```python
from build123d import *

# Parameters (mm, degrees)
SKETCH_1_W                = 82
SKETCH_1_H                = 82
EXTRUDE_1_DEPTH           = 10
SKETCH_4_R                = 10.5
CUT_EXTRUDE_3_DEPTH       = 59.838762733
FILLET_9_R                = 10
HOLE_WIZARD_2_D           = 4.3
HOLE_WIZARD_2_CBORE_D     = 8
HOLE_WIZARD_2_CBORE_DEPTH = 4.6
HOLE_WIZARD_M4_2_D        = 3.3
HOLE_WIZARD_M4_2_DEPTH    = 18.5
HOLE_WIZARD_M4_2_TIP      = 0.991420021
MM_2_D                    = 21.1
HOLE_WIZARD_M4_3_D        = 3.3
HOLE_WIZARD_M6_1_D        = 5
HOLE_WIZARD_M6_2_D        = 5
HOLE_WIZARD_5_0_5_1_D     = 5
HOLE_WIZARD_5_0_5_1_DEPTH = 10
HOLE_WIZARD_5_0_5_1_TIP   = 1.502151548


with BuildPart() as part:
    # 草图1 → 凸台-拉伸1 (new body)
    with BuildSketch(Plane(origin=(0, 0, 0), x_dir=(1, 0, 0), z_dir=(0, 1, 0))):
        Rectangle(SKETCH_1_W, SKETCH_1_H)
    extrude(amount=EXTRUDE_1_DEPTH)

    # 草图4 → 切除-拉伸3 (cut, through all)
    with BuildSketch(Plane(origin=(0, 10, 0), x_dir=(1, 0, 0), z_dir=(0, 1, 0))):
        with Locations(Location((0, -27.5, 0), (0, 0, 270))):
            Circle(SKETCH_4_R)
    extrude(amount=-CUT_EXTRUDE_3_DEPTH, mode=Mode.SUBTRACT)

    # 圆角9
    fillet_9_edges = [part.edges().sort_by_distance(p)[0] for p in [
        (41, 5, 41),
        (-41, 5, 41),
    ]]
    fillet(fillet_9_edges, radius=FILLET_9_R)

    # 打孔尺寸(%根据)开槽圆柱头螺钉的类型2 (through all)
    with Locations(Plane(origin=(0, 10, 0), x_dir=(1, 0, 0), z_dir=(0, 1, 0))):
        with Locations((-16.5, -27.5), (16.5, -27.5)):
            CounterBoreHole(HOLE_WIZARD_2_D / 2, HOLE_WIZARD_2_CBORE_D / 2, HOLE_WIZARD_2_CBORE_DEPTH)

    # M4 螺纹孔2
    with Locations(Plane(origin=(0, 0, -41), x_dir=(-1, 0, 0), z_dir=(0, 0, -1))):
        with Locations((-22.5, 5), (22.5, 5)):
            Hole(HOLE_WIZARD_M4_2_D / 2, depth=HOLE_WIZARD_M4_2_DEPTH)
            with Locations((0, 0, -(HOLE_WIZARD_M4_2_DEPTH + HOLE_WIZARD_M4_2_TIP / 2))):  # 118° drill point
                Cone(0, HOLE_WIZARD_M4_2_D / 2, HOLE_WIZARD_M4_2_TIP, mode=Mode.SUBTRACT)

    # 大小mm 暗销孔2 (through all)
    with Locations(Plane(origin=(0, 10, 0), x_dir=(1, 0, 0), z_dir=(0, 1, 0))):
        with Locations((-25, 13), (25, 13)):
            Hole(MM_2_D / 2)

    # M4 螺纹孔3 (through all)
    with Locations(Plane(origin=(0, 0, 0), x_dir=(-1, 0, 0), z_dir=(0, -1, 0))):
        with Locations((-13.686291501, 24.313708499), (-13.686291501, 1.686291501), (-36.313708499, 1.686291501), (-36.313708499, 24.313708499)):
            hole_wizard_m4_3 = Hole(HOLE_WIZARD_M4_3_D / 2)

    # 镜向2: M4 螺纹孔3 across plane
    add(hole_wizard_m4_3.mirror(Plane(origin=(0, 0, 0), x_dir=(0, 0, 1), z_dir=(1, 0, 0))), mode=Mode.SUBTRACT)

    # M6 螺纹孔1 (through all)
    with Locations(Plane(origin=(0, 10, 0), x_dir=(1, 0, 0), z_dir=(0, 1, 0))):
        with Locations((0, 22)):
            Hole(HOLE_WIZARD_M6_1_D / 2)

    # M6 螺纹孔2 (through all)
    with Locations(Plane(origin=(0, 10, 0), x_dir=(1, 0, 0), z_dir=(0, 1, 0))):
        with Locations((0, -4)):
            Hole(HOLE_WIZARD_M6_2_D / 2)

    # Ø5.0 (5) 直径孔1
    with Locations(Plane(origin=(0, 0, -41), x_dir=(-1, 0, 0), z_dir=(0, 0, -1))):
        with Locations((-32.5, 5), (32.5, 5)):
            Hole(HOLE_WIZARD_5_0_5_1_D / 2, depth=HOLE_WIZARD_5_0_5_1_DEPTH)
            with Locations((0, 0, -(HOLE_WIZARD_5_0_5_1_DEPTH + HOLE_WIZARD_5_0_5_1_TIP / 2))):  # 118° drill point
                Cone(0, HOLE_WIZARD_5_0_5_1_D / 2, HOLE_WIZARD_5_0_5_1_TIP, mode=Mode.SUBTRACT)


solid = part.part
```
Input: part model. Units: mm. Frame: model coordinates. A direction names the side the tool comes from. Round coordinates to 2 decimals unless told otherwise and drop trailing zeros. Loops run counter-clockwise (first coordinate to the right, second up) from the corner with the lowest first, then second, coordinate; pieces in that order, holes last.
1) Pull-direction query (Y, two-part tool) for faces 1 (the flat face through (-14.8, 5.4, 29.2)), 2 (the cylindrical face through (-35.956, 5.07, -22.703)), 3 (the conical face through (-32.9, 4.83, -29.76)); classes: released by +Y, released by -Y, zero draft, split by the parting line, or undercut.
Ans:
face 1: released by +Y
face 2: zero draft
face 3: undercut
2) Material intervals for line 1 (X direction, y = 7.15, z = 27.5); line 2 (X direction, y = 4.3, z = 27.5); line 3 (Z direction, x = -25.5, y = 4.75), sorted ascending.
Ans:
line 1: x = -41 to -20.5, -12.5 to -10.5, 10.5 to 12.5, 20.5 to 41
line 2: x = -41 to -18.65, -14.35 to -10.5, 10.5 to 14.35, 18.65 to 41
line 3: z = -41 to -23.54, -2.46 to 41
3) Section query B-B on x = 0. Return the cut outline in (y, z), plus the area to 3 significant figures.
Ans:
outline: (0, -41) - (10, -41) - (10, -24.5) - (0, -24.5) - close; (0, -19.5) - (10, -19.5) - (10, 1.5) - (0, 1.5) - close; (0, 6.5) - (10, 6.5) - (10, 17) - (0, 17) - close; (0, 38) - (10, 38) - (10, 41) - (0, 41) - close
area: 510 mm2
4) Section query D-D on x = 16.5. Return the cut outline in (y, z), plus the area to 3 significant figures.
Ans:
outline: (0, -41) - (10, -41) - (10, -19.25) - (0, -19.25) - close; (0, -6.75) - (10, -6.75) - (10, 23.5) - (5.4, 23.5) - (5.4, 25.35) - (0, 25.35) - close; (0, 29.65) - (5.4, 29.65) - (5.4, 31.5) - (10, 31.5) - (10, 41) - (0, 41) - close
area: 635 mm2
5) Section query C-C on z = 27.5. Return the cut outline in (x, y).
Ans:
outline: (-41, 0) - (-18.65, 0) - (-18.65, 5.4) - (-20.5, 5.4) - (-20.5, 10) - (-41, 10) - close; (-14.35, 0) - (-10.5, 0) - (-10.5, 10) - (-12.5, 10) - (-12.5, 5.4) - (-14.35, 5.4) - close; (10.5, 0) - (14.35, 0) - (14.35, 5.4) - (12.5, 5.4) - (12.5, 10) - (10.5, 10) - close; (18.65, 0) - (41, 0) - (41, 10) - (20.5, 10) - (20.5, 5.4) - (18.65, 5.4) - close
6) Pin query (flat end, axial travel): pin 1 (6.5 mm diameter, centred on x = 0, z = -22, fed in from +Y); pin 2 (3 mm diameter, centred on x = -36.31, z = -24.31, fed in from -Y); pin 3 (7 mm diameter, centred on x = 16.5, z = 27.5, fed in from +Y). Return the tip coordinate at first contact, or that it passes through.
Ans:
pin 1: stops at y = 10
pin 2: passes through
pin 3: stops at y = 5.4
7) Section query A-A on z = -13. Return the cut outline in (x, y).
Ans:
outline: (-41, 0) - (-35.55, 0) - (-35.55, 10) - (-41, 10) - close; (-14.45, 0) - (14.45, 0) - (14.45, 10) - (-14.45, 10) - close; (35.55, 0) - (41, 0) - (41, 10) - (35.55, 10) - close
8) Set-up query: faces 4 (the cylindrical face through (-38.15, 5.07, 37.99)), 5 (the cylindrical face through (-23.81, 4, -31.72)), 6 (the cylindrical face through (13.55, 7.73, 24.8)). Return all of +Z, -Z, +X, -X, +Y, -Y with unobstructed straight access to the full face (end or side cutting, diameter ignored); none if empty.
Ans:
face 4: +Z, -X, +Y, -Y
face 5: -Z
face 6: +Y
